Check sheet for the modelled part. Datum: model origin and axes. Units: mm. A direction names the side the tool comes from. Round coordinates to 2 decimals unless told otherwise and drop trailing zeros. Order: outer loops, then holes, each group sorted by start corner. A loop starts at its lowest first (then second) coordinate and runs counter-clockwise, first axis right, second up.
from build123d import *

# Parameters (mm, degrees)
BASE_BLOCK_SKETCH_W        = 100
BASE_BLOCK_SKETCH_H        = 63
BASE_BLOCK_100X63X75_DEPTH = 75
TOP_POCKET_SKETCH_W        = 50
TOP_POCKET_SKETCH_H        = 38
TOP_POCKET_38X25X19_DEPTH  = 19
FEET_SKETCH_W              = 32
FEET_SKETCH_H              = 25
FEET_2X_32X25_DEPTH        = 10
SIDE_RIB_DEPTH             = 10


with BuildPart() as part:
    # Base Block Sketch → Base Block 100x63x75 (new body)
    with BuildSketch(Plane(origin=(0, 0, 0), x_dir=(1, 0, 0), z_dir=(0, 1, 0))):
        with Locations((50, 31.5)):
            Rectangle(BASE_BLOCK_SKETCH_W, BASE_BLOCK_SKETCH_H)
    extrude(amount=BASE_BLOCK_100X63X75_DEPTH)

    # Top Pocket Sketch → Top Pocket 38x25x19 (cut)
    with BuildSketch(Plane.XY):
        with Locations((50, 56)):
            Rectangle(TOP_POCKET_SKETCH_W, TOP_POCKET_SKETCH_H)
    extrude(amount=-TOP_POCKET_38X25X19_DEPTH, mode=Mode.SUBTRACT)

    # Feet Sketch → Feet 2x 32x25 (add, symmetric)
    with BuildSketch(Plane.XZ):
        with Locations((16, 12.5)):
            Rectangle(FEET_SKETCH_W, FEET_SKETCH_H)
        with Locations((84, 12.5)):
            Rectangle(FEET_SKETCH_W, FEET_SKETCH_H)
    extrude(amount=FEET_2X_32X25_DEPTH, both=True)

    # Side Rib Sketch → Side Rib (add, symmetric)
    with BuildSketch(Plane(origin=(100, 0, 0), x_dir=(0, 0, -1), z_dir=(1, 0, 0))):
        Polygon((63, 0), (63, 50), (51, 50), (51, -10), (63, -10), align=None)
    extrude(amount=SIDE_RIB_DEPTH, both=True)


solid = part.part
1) Scan lines: line 1 (X direction, y = 0.5, z = 7.5); line 2 (Z direction, x = 5, y = 65.5); line 3 (Y direction, x = 56, z = -56). Record each from-to range of solid material in increasing order.
2) Draft check along X on faces 1 (the face through (0, 32, -28)), 2 (the face through (16, 0, 25)), 3 (the face through (110, 20, -57)), 4 (the face through (75, 56, -9)). Enter one of: pulls with the +X half, pulls with the -X half, needs draft (parallel to the pull), parting line crosses it, or undercut.
3) Sectioned sample at B-B on y = 3.5. Record the cut outline in (x, z).
4) Gauge pin test, flat ends, axial feed: pin 1 (8 mm diameter, centred on x = 27, z = -2, fed in from -Y); pin 2 (5.5 mm diameter, centred on x = 42, z = -7.5, fed in from +Y); pin 3 (11 mm diameter, centred on x = 106, z = -55.5, fed in from +Y); pin 4 (22 mm diameter, centred on y = -2, z = 12, fed in from +X). Record the tip position at first contact, or that the pin passes through.
5) Sectioned sample at D-D on z = -17. Record the cut outline in (x, y).
6) Sectioned sample at C-C on x = 97. Record the cut outline in (y, z).
7) Sectioned sample at A-A on z = 18. Record the cut outline in (x, y).
8) Set-up check for faces 5 (the face through (50, 37, -9)), 6 (the face through (32, 0, 12)), 7 (the face through (16, -5, 0)): record each of +Z, -Z, +X, -X, +Y, -Y from which the full face is reachable in a straight line by a thin tool's end or side.
Values found:
1. line 1: x = 0 to 32, 68 to 100
1. line 2: z = -63 to 0
1. line 3: y = 0 to 75
2. face 1: pulls with the -X half
2. face 2: needs draft
2. face 3: pulls with the +X half
2. face 4: undercut
3. outline: (0, -63) - (110, -63) - (110, -51) - (100, -51) - (100, 25) - (68, 25) - (68, 0) - (32, 0) - (32, 25) - (0, 25) - close
4. pin 1: stops at y = -10
4. pin 2: stops at y = 37
4. pin 3: stops at y = 50
4. pin 4: stops at x = 100
5. outline: (0, 0) - (100, 0) - (100, 75) - (75, 75) - (75, 37) - (25, 37) - (25, 75) - (0, 75) - close
6. outline: (-10, -63) - (75, -63) - (75, 0) - (10, 0) - (10, 25) - (-10, 25) - (-10, 0) - (0, 0) - (0, -51) - (-10, -51) - close
7. outline: (0, -10) - (32, -10) - (32, 10) - (0, 10) - close; (68, -10) - (100, -10) - (100, 10) - (68, 10) - close
8. face 5: +Z, +Y
8. face 6: +Z, +Y, -Y
8. face 7: -Z, +X, -X, -Y
